Read the model definition and answer for the solid it produces. Units are mm, in the model's axes. A direction names the side the tool comes from. Round coordinates to 2 decimals unless told otherwise and drop trailing zeros. Order: outer loops, then holes, each group sorted by start corner. A loop starts at its lowest first (then second) coordinate and runs counter-clockwise, first axis right, second up.
from build123d import *

# Parameters (mm, degrees)
BASE_PROFILE_SKETCH_R    = 12.5
BASE_BODY_DEPTH          = 36
SLOT_CUT_DEPTH           = 118
ARM_PROFILE_SKETCH_R     = 57.5
ARM_PROFILE_SKETCH_R_2   = 37.5
ARM_BOSS_DEPTH           = 60
ARM_BOSS_REGION_2_DEPTH  = 55
HUB_SKETCH_R             = 37.5
HUB_SKETCH_R_2           = 22.5
HUB_BOSS_DEPTH           = 25
SUPPORT_WEB_DEPTH        = 12.5
PAD_SKETCH_60X60_R       = 30
PAD_SKETCH_60X60_R_2     = 12.5
MOUNTING_PAD_60X60_DEPTH = 3


with BuildPart() as part:
    # Base Profile Sketch → Base Body (new body)
    with BuildSketch(Plane.XY):
        with BuildLine():
            Line((-66.25, 55), (19.208333333, 55))
            ThreePointArc((19.208333333, 55), (55.208333333, 91), (91.208333333, 55))
            Line((91.208333333, 55), (91.208333333, -55))
            ThreePointArc((91.208333333, -55), (55.208333333, -91), (19.208333333, -55))
            Line((19.208333333, -55), (-66.25, -55))
            Line((-66.25, -55), (-66.25, 55))
        make_face()
        with Locations((55.208333333, 55)):
            Circle(BASE_PROFILE_SKETCH_R, mode=Mode.SUBTRACT)
        with Locations((55.208333333, -55)):
            Circle(BASE_PROFILE_SKETCH_R, mode=Mode.SUBTRACT)
    extrude(amount=BASE_BODY_DEPTH)

    # Slot Sketch → Slot Cut (cut, symmetric)
    with BuildSketch(Plane(origin=(0, 0, 0), x_dir=(1, 0, 0), z_dir=(0, 1, 0))):
        Polygon((-8.75, -36), (-8.75, -30), (91.208333333, -30), (91.208333333, -36), (19.208333333, -36), align=None)
    extrude(amount=SLOT_CUT_DEPTH, both=True, mode=Mode.SUBTRACT)



with BuildPart() as body_2:
    # Arm Profile Sketch → Arm Boss (new, symmetric)
    with BuildSketch(Plane(origin=(0, 0, 0), x_dir=(1, 0, 0), z_dir=(0, 1, 0))):
        with Locations(Location((-8.75, 130, 0), (0, 0, 270))):
            Circle(ARM_PROFILE_SKETCH_R)
        with Locations(Location((-8.75, 130, 0), (0, 0, 270))):
            Circle(ARM_PROFILE_SKETCH_R_2, mode=Mode.SUBTRACT)
    extrude(amount=ARM_BOSS_DEPTH, both=True)


with BuildPart() as part_1:
    add(part.part)

    add(body_2.part)  # Arm Boss Region 2 merges body 2
    # Sketch4_3 → Arm Boss Region 2 (add, symmetric)
    with BuildSketch(Plane(origin=(0, 0, 0), x_dir=(1, 0, 0), z_dir=(0, 1, 0))):
        with BuildLine():
            Line((-66.25, 130), (-66.25, 0))
            Line((-66.25, 0), (-36.25, 0))
            Line((-36.25, 0), (-36.25, 79.502475308))
            ThreePointArc((-36.25, 79.502475308), (-58.184299833, 100.631649689), (-66.25, 130))
        make_face()
    extrude(amount=ARM_BOSS_REGION_2_DEPTH, both=True)



with BuildPart() as body_2_2:
    # Hub Sketch → Hub Boss (new, symmetric)
    with BuildSketch(Plane(origin=(0, 0, 0), x_dir=(1, 0, 0), z_dir=(0, 1, 0))):
        with Locations(Location((-118.75, 39, 0), (0, 0, 270))):
            Circle(HUB_SKETCH_R)
        with Locations(Location((-118.75, 39, 0), (0, 0, 270))):
            Circle(HUB_SKETCH_R_2, mode=Mode.SUBTRACT)
    extrude(amount=HUB_BOSS_DEPTH, both=True)


with BuildPart() as part_2:
    add(part_1.part)

    add(body_2_2.part)  # Support Web merges body 2 2
    # Web Sketch → Support Web (add, symmetric)
    with BuildSketch(Plane(origin=(0, 0, 0), x_dir=(1, 0, 0), z_dir=(0, 1, 0))):
        with BuildLine():
            Line((-146.465572764, 64.260582462), (-51.247211572, 168.732893109))
            ThreePointArc((-51.247211572, 168.732893109), (-62.368278905, 150.768489769), (-66.25, 130))
            Line((-66.25, 130), (-66.25, -36))
            Line((-66.25, -36), (-137.966934712, 6.798145701))
            ThreePointArc((-137.966934712, 6.798145701), (-81.653531514, 44.486531314), (-146.465572764, 64.260582462))
        make_face()
    extrude(amount=SUPPORT_WEB_DEPTH, both=True)

    # Pad Sketch 60x60 → Mounting Pad 60x60 (add, symmetric)
    # profile 1 of 2: a face of its own
    with BuildSketch(Plane(origin=(0, 0, 0), x_dir=(-1, 0, 0), z_dir=(0, 0, -1))):
        with Locations(Location((-55.208333333, 55, 0), (0, 0, 180))):
            Circle(PAD_SKETCH_60X60_R)
        with Locations((-55.208333333, 55)):
            Circle(PAD_SKETCH_60X60_R_2, mode=Mode.SUBTRACT)
    # profile 2 of 2: a face of its own
    with BuildSketch(Plane(origin=(0, 0, 0), x_dir=(-1, 0, 0), z_dir=(0, 0, -1))):
        with Locations(Location((-55.208333333, -55, 0), (0, 0, 180))):
            Circle(PAD_SKETCH_60X60_R)
        with Locations((-55.208333333, -55)):
            Circle(PAD_SKETCH_60X60_R_2, mode=Mode.SUBTRACT)
    extrude(amount=MOUNTING_PAD_60X60_DEPTH, both=True)


solid = part_2.part
Q1. A cutting plane is placed at B-B, the plane y = -9. Give the vertices of the cut face in (x, z), plus the area to 3 significant figures.
Outcome:
outline: (-146.47, -64.26) - (-51.25, -168.73) arc R57.5 ccw (long way) to (-36.25, -79.5) - (-36.25, 0) - (91.21, 0) - (91.21, 30) - (-8.75, 30) - (-8.75, 36) - (-66.25, 36) - (-137.97, -6.8) arc R37.5 ccw to start; hole circle Ø45 at (-118.75, -39); hole circle Ø75 at (-8.75, -130)
area: 22,300 mm2
Q2. A cutting plane is placed at D-D, the plane y = -39. Give the vertices of the cut face in (x, z).
Outcome:
outline: (-66.25, -130) arc R57.5 ccw (long way) to (-36.25, -79.5) - (-36.25, 0) - (29.83, 0) - (29.83, -3) - (80.59, -3) - (80.59, 0) - (91.21, 0) - (91.21, 30) - (-8.75, 30) - (-8.75, 36) - (-66.25, 36) - close; hole circle Ø75 at (-8.75, -130)
Q3. Straight lines are drawn through the part: probe 1 along Z at (x, y) = (-8, 2); probe 2 along X at (y, z) = (8, -39); probe 3 along Z at (x, y) = (-31.5, -14). For each, find the intervals that lie inside material, in ascending order.
Outcome:
probe 1: z = -187.5 to -167.49, -92.51 to -72.5, 0 to 30
probe 2: x = -156.25 to -141.25, -96.25 to -36.25
probe 3: z = -182.81 to -159.81, -100.19 to -77.19, 0 to 36
Q4. A cutting plane is placed at C-C, the plane x = -101. Give the vertices of the cut face in (y, z).
Outcome:
outline: (-25, -72.03) - (-12.5, -72.03) - (-12.5, -114.14) - (12.5, -114.14) - (12.5, -72.03) - (25, -72.03) - (25, -52.83) - (-25, -52.83) - close; (-25, -25.17) - (25, -25.17) - (25, -5.97) - (12.5, -5.97) - (12.5, 15.26) - (-12.5, 15.26) - (-12.5, -5.97) - (-25, -5.97) - close
Q5. For a pull along X with two mould halves and no side action, classify faces 1 (the face through (-81, -12.5, -59)), 2 (the face through (-43, 55, -11)), 3 (the face through (-152.02, 0.35, -21.7)), 4 (the face through (54.42, 90.99, 14.79)) as released by +X, released by -X, zero draft, split by the parting line, or undercut.
Outcome:
face 1: undercut
face 2: zero draft
face 3: undercut
face 4: split by the parting line
Q6. A cutting plane is placed at A-A, the plane z = -39. Give the vertices of the cut face in (x, y), plus the area to 4 significant figures.
Outcome:
outline: (-156.25, -25) - (-141.25, -25) - (-141.25, 25) - (-156.25, 25) - close; (-96.25, -25) - (-81.25, -25) - (-81.25, -12.5) - (-66.25, -12.5) - (-66.25, -55) - (-36.25, -55) - (-36.25, 55) - (-66.25, 55) - (-66.25, 12.5) - (-81.25, 12.5) - (-81.25, 25) - (-96.25, 25) - close
area: 5,175 mm2
Q7. For faces 5 (the face through (68, -55, -3)), 6 (the face through (41, 1, 30)), 7 (the face through (-66.25, 34, -48)), 8 (the face through (-66.25, -33, -48)), 9 (the face through (82.92, 66.49, -1.48)), determine the directions among +Z, -Z, +X, -X, +Y, -Y from which every point of the face is accessible in a straight line to the end or side of a thin tool.
Outcome:
face 5: +X, +Y, -Y
face 6: +Z, +X, +Y, -Y
face 7: +Z, -Z, +Y
face 8: +Z, -Z, -Y
face 9: none
Q8. Flat-ended cylindrical pins translate along their axes: pin 1 (5 mm diameter, centred on y = -35, z = -34, fed in from -X); pin 2 (12 mm diameter, centred on x = -29.5, z = -81, fed in from -Y); pin 3 (24 mm diameter, centred on y = 13.5, z = -22.5, fed in from +X). Find the tip coordinate at first contact, or state that the pin passes through.
Outcome:
pin 1: stops at x = -66.25
pin 2: stops at y = -60
pin 3: stops at x = -36.25
